Design review of the part built by this model. Coordinates are the model's own, in mm. Face numbers are marked on the shaded views. Give positions to 0.01 mm unless a question says otherwise; leave off trailing zeros. Loops run counter-clockwise (first coordinate to the right, second up) from the corner with the lowest first, then second, coordinate; pieces in that order, holes last. Notation, with made-up numbers: (65, -35) -> (76, -35) arc R13 ccw to (76, -18) -> close; hole circle Ø3 at (87.5, 47.5). An arc over 180 degrees is marked (long way). Use CSV: the item, a comma, the result in double quotes. Start each with the question number.
Item 1: We need section C-C (z = 22). State the section outline as (x, y) points.
Item 2: We need section A-A (x = 6). State the section outline as (y, z) points, plus the area to 3 significant figures.
Item 3: Clearance check with flat-ended pins moving along their axes: pin 1 (3 mm diameter, centred on x = 1, y = 1, fed in from +Z); pin 2 (8 mm diameter, centred on x = 21, y = 5.5, fed in from +Z). State where each tip first meets the part, or that it passes through.
Item 4: We need section D-D (x = 19). State the section outline as (y, z) points, plus the area to 3 significant figures.
Item 5: The part is to be moulded in two halves that separate along Y. For the marked faces 1, 2, 3 and 4, say which applies: +Y half, -Y half, draft (parallel to the pull), parting line (faces both ways), or undercut.
Item 6: We need section B-B (y = -0.75). State the section outline as (x, z) points.
Item 7: Wall thickness on line 1 along Y through (x, z) = (1, 22.25); line 2 along Z through (x, y) = (-5.5, -0.5); line 3 along X through (y, z) = (-8, 18.25): over which ranges is each line inside the solid? List them lowest first. Write a range as from..to.
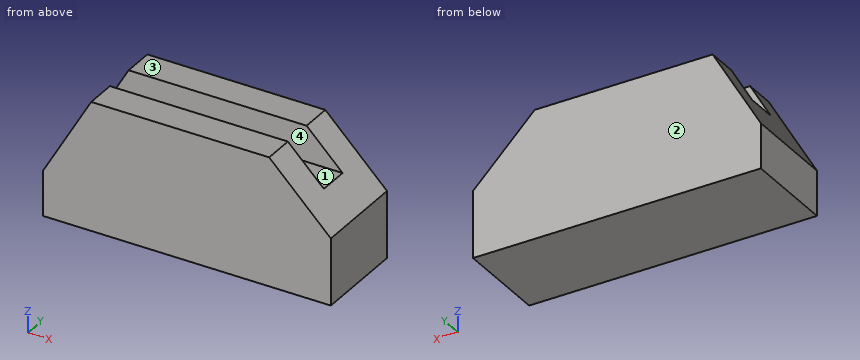
from build123d import *

# Parameters (mm, degrees)
BASE_PROFILE_SKETCH_W    = 56
BASE_PROFILE_SKETCH_H    = 18
BASE_BLOCK_DEPTH         = 25
ANGLED_CORNER_CUTS_DEPTH = 42.629316593
SLOT_SKETCH_W            = 47
SLOT_SKETCH_H            = 6
SLOT_47X6_DEPTH          = 7


with BuildPart() as part:
    # Base Profile Sketch → Base Block (new body)
    with BuildSketch(Plane.XY):
        Rectangle(BASE_PROFILE_SKETCH_W, BASE_PROFILE_SKETCH_H)
    extrude(amount=BASE_BLOCK_DEPTH)

    # Corner Cut Sketch → Angled Corner Cuts (cut, through all)
    with BuildSketch(Plane.XZ.offset(9)):
        Polygon((28, 13), (16, 25), (28, 25), align=None)
        Polygon((-28, 13), (-28, 8.753100352), (-18.619848115, 25), (-28, 25), align=None)
    extrude(amount=-ANGLED_CORNER_CUTS_DEPTH, mode=Mode.SUBTRACT)

    # Slot Sketch → Slot 47x6 (cut)
    with BuildSketch(Plane.XY.offset(25)):
        Rectangle(SLOT_SKETCH_W, SLOT_SKETCH_H)
    extrude(amount=-SLOT_47X6_DEPTH, mode=Mode.SUBTRACT)


solid = part.part
Results found:
1,outline,"(-20.35, -9) -> (19, -9) -> (19, -3) -> (-20.35, -3) -> close; (-20.35, 3) -> (19, 3) -> (19, 9) -> (-20.35, 9) -> close"
2,outline,"(-9, 0) -> (9, 0) -> (9, 25) -> (3, 25) -> (3, 18) -> (-3, 18) -> (-3, 25) -> (-9, 25) -> close"
2,area,"408 mm²"
3,pin 1,"z = 18"
3,pin 2,"z = 24"
4,outline,"(-9, 0) -> (9, 0) -> (9, 22) -> (3, 22) -> (3, 18) -> (-3, 18) -> (-3, 22) -> (-9, 22) -> close"
4,area,"372 mm²"
5,face 1,"undercut"
5,face 2,"+Y half"
5,face 3,"draft"
5,face 4,"undercut"
6,outline,"(-28, 0) -> (28, 0) -> (28, 13) -> (23, 18) -> (-22.66, 18) -> (-28, 8.75) -> close"
7,line 1,"-9..-3, 3..9"
7,line 2,"0..18"
7,line 3,"-22.52..22.75"
